```python
from build123d import *

# Parameters (mm, degrees)
SKETCH_1_W                   = 20
SKETCH_1_H                   = 23
EXTRUDE_1_DEPTH              = 22
HOLE_WIZARD_M6_1_D           = 6.6
HOLE_WIZARD_M6_1_DEPTH       = 22.25
HOLE_WIZARD_M6_1_CBORE_D     = 11
HOLE_WIZARD_M6_1_CBORE_DEPTH = 15
HOLE_WIZARD_M6_1_TIP         = 1.982840043
CHAMFER_1_SIZE               = 1


with BuildPart() as part:
    # 草图1 → 凸台-拉伸1 (new body)
    with BuildSketch(Plane(origin=(0, 0, 0), x_dir=(1, 0, 0), z_dir=(0, 1, 0))):
        Rectangle(SKETCH_1_W, SKETCH_1_H)
    extrude(amount=EXTRUDE_1_DEPTH)

    # M6 六角凹头螺钉的柱形沉头孔1
    with Locations(Plane(origin=(0, 0, 0), x_dir=(-1, 0, 0), z_dir=(0, -1, 0))):
        with Locations((0, 0)):
            CounterBoreHole(HOLE_WIZARD_M6_1_D / 2, HOLE_WIZARD_M6_1_CBORE_D / 2, HOLE_WIZARD_M6_1_CBORE_DEPTH, depth=HOLE_WIZARD_M6_1_DEPTH)
            with Locations((0, 0, -(HOLE_WIZARD_M6_1_DEPTH + HOLE_WIZARD_M6_1_TIP / 2))):  # 118° drill point
                Cone(0, HOLE_WIZARD_M6_1_D / 2, HOLE_WIZARD_M6_1_TIP, mode=Mode.SUBTRACT)

    # 倒角1
    chamfer_1_edges = [part.edges().sort_by_distance(p)[0] for p in [
        (10, 11, 11.5),
        (-10, 11, 11.5),
        (-10, 11, -11.5),
        (10, 11, -11.5),
    ]]
    chamfer(chamfer_1_edges, length=CHAMFER_1_SIZE)


solid = part.part
```
The model under review builds one solid part; all positions refer to its coordinate system, in mm. Give positions to 0.01 mm unless a question says otherwise; leave off trailing zeros. Order: outer loops, then holes, each group sorted by start corner. A loop starts at its lowest first (then second) coordinate and runs counter-clockwise, first axis right, second up. Notation, with made-up numbers: (44.5, 84) - (91.5, 84) arc R12 cw to (91.5, 104) - close; hole circle Ø2 at (87.5, -26). An arc over 180 degrees is marked (long way). Use CSV: the item, a comma, the result in double quotes. Start each with the question number.
Q1. To check wall thickness, follow line 1 along Z through (x, y) = (0, 10.75); line 2 along Z through (x, y) = (0, 18.25); line 3 along X through (y, z) = (20.25, -1.5). State the ranges of each line that lie inside material, in increasing order. Write a range as [from, to].
Q2. We need section A-A, the plane z = 0. Write out the cut boundary in (x, y).
Q3. We need section B-B, the plane x = 0. Write out the cut boundary in (y, z), and give its area (3 significant figures).
Q4. The part is to be moulded in two halves that separate along X. For faces 1 (the flat face through (-4, 15, 0)), 2 (the cylindrical face through (1.19, 7.4, 5.37)), 3 (the flat face through (9.5, 10.8, 11)), 4 (the flat face through (-10, 11, 0)), say which applies: +X half, -X half, draft (parallel to the pull), parting line (faces both ways), or undercut.
Q5. Clearance check with a flat-ended pin moving along its axis: pin 1 Ø4 at (x, z) = (-0.5, 9) entering from -Y. State where the tip first meets the part, or that it passes through.
Q6. We need section D-D, the plane x = 3.75. Write out the cut boundary in (y, z).
Q7. We need section C-C, the plane y = 19.5. Write out the cut boundary in (x, z), and give its area (3 significant figures).
Outcome:
1,line 1,"z = [-11.5, -5.5], [5.5, 11.5]"
1,line 2,"z = [-11.5, -3.3], [3.3, 11.5]"
1,line 3,"x = [-10, -2.94], [2.94, 10]"
2,outline,"(-10, 0) - (-5.5, 0) - (-5.5, 15) - (-3.3, 15) - (-3.3, 22) - (-10, 22) - close; (3.3, 15) - (5.5, 15) - (5.5, 0) - (10, 0) - (10, 22) - (3.3, 22) - close"
3,outline,"(0, -11.5) - (22, -11.5) - (22, -3.3) - (15, -3.3) - (15, -5.5) - (0, -5.5) - close; (0, 5.5) - (15, 5.5) - (15, 3.3) - (22, 3.3) - (22, 11.5) - (0, 11.5) - close"
3,area,"295 mm^2"
4,face 1,"undercut"
4,face 2,"undercut"
4,face 3,"+X half"
4,face 4,"-X half"
5,pin 1,"stops at y = 0"
6,outline,"(0, -11.5) - (22, -11.5) - (22, 11.5) - (0, 11.5) - (0, 4.02) - (15, 4.02) - (15, -4.02) - (0, -4.02) - close"
7,outline,"(-10, -10.5) - (-9, -11.5) - (9, -11.5) - (10, -10.5) - (10, 10.5) - (9, 11.5) - (-9, 11.5) - (-10, 10.5) - close; hole circle Ø6.6 at (0, 0)"
7,area,"424 mm^2"
